Geometry: final body of the model. Coordinates: model frame, mm. A direction names the side the tool comes from. Coordinates: 2 decimals unless noted, no trailing zeros. Loops run counter-clockwise (first coordinate to the right, second up) from the corner with the lowest first, then second, coordinate; pieces in that order, holes last. Notation, with made-up numbers: (8, 30) - (29, 30) arc R30 ccw to (29, 66) - close; hole circle Ø1 at (11.25, -11.75). An arc over 180 degrees is marked (long way). Return JSON: item names as keys, results as strings.
from build123d import *

# Parameters (mm, degrees)
L_BRACKET_BASE_DEPTH                      = 48
BASE_CORNER_ROUNDS_R16_R                  = 16
SLOT_CUT_DEPTH                            = 48
BACK_PLATE_SKETCH_W                       = 48
BACK_PLATE_SKETCH_H                       = 38
BACK_PLATE_SKETCH_R                       = 4.5
BACK_PLATE_WITH_MOUNTING_HOLES_2X_9_DEPTH = 9
BEARING_HUB_SKETCH_R                      = 12
BEARING_HUB_SKETCH_R_2                    = 8
BEARING_HUB_DEPTH                         = 9
SUPPORT_RIB_DEPTH                         = 4
BEARING_BORE_SKETCH_R                     = 8
BEARING_BORE_16_DEPTH                     = 90.693923986
BACK_PLATE_CORNER_ROUNDS_R9_R             = 9


with BuildPart() as part:
    # L Bracket Profile Sketch → L Bracket Base (new body)
    with BuildSketch(Plane.XY):
        Polygon((0, 0), (39, 0), (39, 3), (60, 3), (60, 0), (60, -28), (69, -28), (69, 12), (0, 12), align=None)
    extrude(amount=-L_BRACKET_BASE_DEPTH)

    # Base Corner Rounds R16
    base_corner_rounds_r16_edges = [part.edges().sort_by_distance(p)[0] for p in [
        (64.5, -28, 0),
        (64.5, -28, -48),
    ]]
    fillet(base_corner_rounds_r16_edges, radius=BASE_CORNER_ROUNDS_R16_R)

    # Slot Sketch → Slot Cut (cut)
    with BuildSketch(Plane(origin=(69, 0, 0), x_dir=(0, 0, -1), z_dir=(1, 0, 0))):
        with BuildLine():
            Line((15, -10.5), (33, -10.5))
            ThreePointArc((33, -10.5), (37.5, -15), (33, -19.5))
            Line((33, -19.5), (15, -19.5))
            ThreePointArc((15, -19.5), (10.5, -15), (15, -10.5))
        make_face()
    extrude(amount=-SLOT_CUT_DEPTH, mode=Mode.SUBTRACT)

    # Back Plate Sketch → Back Plate with Mounting Holes 2xØ9 (add)
    with BuildSketch(Plane.ZY):
        with Locations((-24, 31)):
            Rectangle(BACK_PLATE_SKETCH_W, BACK_PLATE_SKETCH_H)
        with Locations((-39, 32)):
            Circle(BACK_PLATE_SKETCH_R, mode=Mode.SUBTRACT)
        with Locations((-9, 32)):
            Circle(BACK_PLATE_SKETCH_R, mode=Mode.SUBTRACT)
    extrude(amount=-BACK_PLATE_WITH_MOUNTING_HOLES_2X_9_DEPTH)



with BuildPart() as body_2:
    # Bearing Hub Sketch → Bearing Hub (new, symmetric)
    with BuildSketch(Plane.XY.offset(-24)):
        with Locations((39, 32)):
            Circle(BEARING_HUB_SKETCH_R)
        with Locations((39, 32)):
            Circle(BEARING_HUB_SKETCH_R_2, mode=Mode.SUBTRACT)
    extrude(amount=BEARING_HUB_DEPTH, both=True)


with BuildPart() as part_1:
    add(part.part)

    add(body_2.part)  # Support Rib merges body 2
    # Support Rib Sketch → Support Rib (add, symmetric)
    with BuildSketch(Plane.XY.offset(-24)):
        with BuildLine():
            Line((69, 12), (48.6, 39.2))
            ThreePointArc((48.6, 39.2), (44.276884864, 42.553769728), (39, 44))
            Line((39, 44), (15, 44))
            ThreePointArc((15, 44), (10.757359313, 45.757359313), (9, 50))
            Line((9, 50), (9, 12))
            Line((9, 12), (69, 12))
        make_face()
    extrude(amount=SUPPORT_RIB_DEPTH, both=True)

    # Bearing Bore Sketch → Bearing Bore Ø16 (cut, through all)
    with BuildSketch(Plane.XY.offset(-20)):
        with Locations((39, 32)):
            Circle(BEARING_BORE_SKETCH_R)
    extrude(amount=-BEARING_BORE_16_DEPTH, mode=Mode.SUBTRACT)

    # Back Plate Corner Rounds R9
    back_plate_corner_rounds_r9_edges = [part_1.edges().sort_by_distance(p)[0] for p in [
        (4.5, 50, -48),
        (4.5, 50, 0),
    ]]
    fillet(back_plate_corner_rounds_r9_edges, radius=BACK_PLATE_CORNER_ROUNDS_R9_R)


solid = part_1.part
Item 1: First-contact query: pin 1 Ø2 at (y, z) = (41, -20) entering from +X; pin 2 Ø11.5 at (x, z) = (23, -27) entering from -Y; pin 3 Ø19 at (x, y) = (34, 28) entering from +Z; pin 4 Ø5.5 at (y, z) = (32, -9) entering from -X. Flat tips, straight axial feed; report the tip coordinate or a pass-through.
Worked out:
{"pin 1": "x = 47.94", "pin 2": "y = 0", "pin 3": "z = -15", "pin 4": "through"}
Item 2: Section query C-C, the plane x = 8. Return loops of the section in (y, z).
Worked out:
{"outline": "(0, -48) - (41, -48) arc R9 ccw to (50, -39) - (50, -9) arc R9 ccw to (41, 0) - (0, 0) - close; hole circle Ø9 at (32, -39); hole circle Ø9 at (32, -9)"}
Item 3: Ray query, probe 1 along X at (y, z) = (32, -30.2); probe 2 along X at (y, z) = (30.5, -18.5); probe 3 along Y at (x, z) = (7.25, -39). Return the intervals inside material, ascending. Write a range as from..to.
Worked out:
{"probe 1": "0..9, 27..31, 47..51", "probe 2": "0..9, 27.09..31.14, 46.86..50.91", "probe 3": "0..27.5, 36.5..50"}
Item 4: Section query A-A, the plane y = 32. Return loops of the section in (x, z).
Worked out:
{"outline": "(0, -48) - (9, -48) - (9, -43.5) - (0, -43.5) - close; (0, -34.5) - (9, -34.5) - (9, -28) - (27, -28) - (27, -33) - (31, -33) - (31, -15) - (27, -15) - (27, -20) - (9, -20) - (9, -13.5) - (0, -13.5) - close; (0, -4.5) - (9, -4.5) - (9, 0) - (0, 0) - close; (47, -33) - (51, -33) - (51, -28) - (54, -28) - (54, -20) - (51, -20) - (51, -15) - (47, -15) - close"}
Item 5: Section query D-D, the plane z = -8. Return loops of the section in (x, y), and give its area (3 significant figures).
Worked out:
{"outline": "(0, 0) - (39, 0) - (39, 3) - (60, 3) - (60, -25.86) - (69, -25.86) - (69, 12) - (9, 12) - (9, 27.61) - (0, 27.61) - close; (0, 36.39) - (9, 36.39) - (9, 49.94) - (0, 49.94) - close", "area": "1,260 mm^2"}
Item 6: Section query B-B, the plane z = -27. Return loops of the section in (x, y).
Worked out:
{"outline": "(0, 0) - (39, 0) - (39, 3) - (60, 3) - (60, -10.5) - (69, -10.5) - (69, 12) - (48.6, 39.2) arc R12 ccw to (39, 44) - (15, 44) arc R6 cw to (9, 50) - (0, 50) - close; (60, -28) - (69, -28) - (69, -19.5) - (60, -19.5) - close; hole circle Ø16 at (39, 32)"}
Item 7: Reachability of faces 1 (the face through (19, 0, -24)), 2 (the face through (47, 30, -33)), 3 (the face through (49, 3, -24)), 4 (the face through (64.6, -14.9, -37.5)) from +Z, -Z, +X, -X, +Y, -Y: full face, straight path, thin tool, end or side. Return the list, or none.
Worked out:
{"face 1": "+Z, -Z, -X, -Y", "face 2": "-Z, +X, +Y", "face 3": "+Z, -Z, -Y", "face 4": "+X, -X"}
Item 8: Mould query, pull axis Z, two halves, no side actions, for faces 5 (the face through (4, 50, -24)), 6 (the face through (64.6, -15.1, -10.5)), 7 (the face through (65, -19.5, -24)), 8 (the face through (25, 27, -28)). Classes: +Z half, -Z half, draft (parallel to the pull), parting line (faces both ways), or undercut.
Worked out:
{"face 5": "draft", "face 6": "undercut", "face 7": "undercut", "face 8": "-Z half"}
